Part model, mm, in its own coordinate system. A direction names the side the tool comes from. Coordinates: 2 decimals unless noted, no trailing zeros. Write each loop counter-clockwise with the first axis right and the second up, starting at its lowest first coordinate (ties: lowest second). Pieces come first, ordered by that corner, then holes. Notation, with made-up numbers: (81.5, 64) -> (136.5, 64) arc R27 cw to (136.5, 90) -> close; hole circle Ø4 at (21, 44.5). An arc over 180 degrees is marked (long way). Write item = value, one per line. Start each with the question number.
Q1. Band-saw the part on D-D, the plane x = 127. List the corners of the cut face in (y, z).
Q2. Band-saw the part on C-C, the plane x = 62. List the corners of the cut face in (y, z), plus the area to 3 significant figures.
Q3. Pull direction X, two halves, no side cores. Call faces 3 (the flat face through (45, 0, 0)), 4 (the cylindrical face through (25.344, 11.126, -19.936)), 5 (the cylindrical face through (66.6, 9.9, 35)): released by +X, released by -X, zero draft, split by the parting line, or undercut.
Q4. Pin check, flat tips, straight feed: P1, Ø5, axis at y = 13.5, z = 15.5, coming from the -X side; P2, Ø5, axis at x = 10.5, y = 7.5, coming from the -Z side; P3, Ø1.5, axis at x = 114, y = 17, coming from the +Z side; P4, Ø8, axis at x = 19, z = -3.5, coming from the -Y side. Stop position of each tip, or through.
Q5. Band-saw the part on A-A, the plane z = 0. List the corners of the cut face in (x, y), plus the area to 3 significant figures.
Q6. Band-saw the part on B-B, the plane y = 10.5. List the corners of the cut face in (x, z).
Q7. Tool access for faces 1 (the cylindrical face through (105.758, 11.126, 19.618)), 2 (the cylindrical face through (143.727, 0.986, -0.976)): list every direction of +Z, -Z, +X, -X, +Y, -Y with a clear straight run to the whole face (end or side of a thin tool).
Q8. Probe line 1 (X direction, y = 1.25, z = 0); line 2 (X direction, y = 7.5, z = 0); line 3 (Z direction, x = 64.5, y = 13). List the from-to ranges inside material, lowest first.
from build123d import *

# Parameters (mm, degrees)
PLATE_OUTLINE_AND_HOLES_SKETCH_R   = 7.5
PLATE_OUTLINE_AND_HOLES_SKETCH_R_2 = 20
PLATE_BODY_20MM_DEPTH              = 20
POCKET_18MM_DEEP_DEPTH             = 18


with BuildPart() as part:
    # Plate Outline and Holes Sketch → Plate Body 20mm (new body)
    with BuildSketch(Plane(origin=(0, 0, 0), x_dir=(1, 0, 0), z_dir=(0, 1, 0))):
        with BuildLine():
            ThreePointArc((0, -19.652996117), (25.514601751, -22.586747832), (49.820562895, -30.88265372))
            ThreePointArc((49.820562895, -30.88265372), (51.138080036, -31.506466617), (52.447922151, -32.146238124))
            ThreePointArc((52.447922151, -32.146238124), (66.786580153, -34.996485409), (81.03870417, -31.741030931))
            ThreePointArc((81.03870417, -31.741030931), (82.081542873, -31.206935864), (83.12954659, -30.683048174))
            ThreePointArc((83.12954659, -30.683048174), (105.326078872, -22.335617103), (128.730725009, -18.516168186))
            ThreePointArc((128.730725009, -18.516168186), (156.18959255, -2.007382475), (132.581174315, 19.652996117))
            ThreePointArc((132.581174315, 19.652996117), (106.605286262, 22.709869626), (81.908714055, 31.322102615))
            ThreePointArc((81.908714055, 31.322102615), (81.473287731, 31.530691668), (81.03870417, 31.741030931))
            ThreePointArc((81.03870417, 31.741030931), (66.786580153, 34.996485409), (52.447922151, 32.146238124))
            ThreePointArc((52.447922151, 32.146238124), (51.138080036, 31.506466617), (49.820562895, 30.88265372))
            ThreePointArc((49.820562895, 30.88265372), (25.514601751, 22.586747832), (0, 19.652996117))
            ThreePointArc((0, 19.652996117), (-23.709412843, 0), (0, -19.652996117))
        make_face()
        with Locations(Location((-3.709412843, 0, 0), (0, 0, 270))):
            Circle(PLATE_OUTLINE_AND_HOLES_SKETCH_R, mode=Mode.SUBTRACT)
        with Locations(Location((66.290587157, 0, 0), (0, 0, 270))):
            Circle(PLATE_OUTLINE_AND_HOLES_SKETCH_R_2, mode=Mode.SUBTRACT)
        with Locations(Location((136.290587157, 0, 0), (0, 0, 270))):
            Circle(PLATE_OUTLINE_AND_HOLES_SKETCH_R, mode=Mode.SUBTRACT)
    extrude(amount=PLATE_BODY_20MM_DEPTH)

    # Pocket Outline Sketch → Pocket 18mm Deep (cut)
    with BuildSketch(Plane(origin=(0, 20, 0), x_dir=(1, 0, 0), z_dir=(0, 1, 0))):
        with BuildLine():
            ThreePointArc((0, 16.772992409), (-20.887684525, 0), (0, -16.772992409))
            ThreePointArc((0, -16.772992409), (24.982456418, -19.938077439), (49.092914173, -27.206276583))
            ThreePointArc((49.092914173, -27.206276583), (66.290587157, -32.186044206), (83.488260142, -27.206276583))
            ThreePointArc((83.488260142, -27.206276583), (106.082407894, -19.537899767), (129.668226583, -15.931146045))
            ThreePointArc((129.668226583, -15.931146045), (153.543328212, 0), (129.668226583, 15.931146045))
            ThreePointArc((129.668226583, 15.931146045), (106.363417967, 20.688843047), (83.488260142, 27.206276583))
            ThreePointArc((83.488260142, 27.206276583), (66.290587157, 32.186044206), (49.092914173, 27.206276583))
            ThreePointArc((49.092914173, 27.206276583), (24.998686698, 19.861707266), (0, 16.772992409))
        make_face()
    extrude(amount=-POCKET_18MM_DEEP_DEPTH, mode=Mode.SUBTRACT)


solid = part.part
Ans:
q1.outline = (0, -19.83) -> (20, -19.83) -> (20, -16.38) -> (2, -16.38) -> (2, 16.13) -> (20, 16.13) -> (20, 18.64) -> (0, 18.64) -> close
q2.outline = (0, -34.74) -> (20, -34.74) -> (20, -31.9) -> (2, -31.9) -> (2, -19.53) -> (0, -19.53) -> close; (0, 19.53) -> (2, 19.53) -> (2, 31.9) -> (20, 31.9) -> (20, 34.74) -> (0, 34.74) -> close
q2.area = 163 mm2
q3.face_3 = zero draft
q3.face_4 = undercut
q3.face_5 = split by the parting line
q4.P1 = -18.91
q4.P2 = -20.45
q4.P3 = 20.51
q4.P4 = 0
q5.outline = (-23.71, 0) -> (-11.21, 0) -> (-11.21, 2) -> (-20.89, 2) -> (-20.89, 20) -> (-23.71, 20) -> close; (3.79, 0) -> (46.29, 0) -> (46.29, 2) -> (3.79, 2) -> close; (86.29, 0) -> (128.79, 0) -> (128.79, 2) -> (86.29, 2) -> close; (143.79, 0) -> (156.29, 0) -> (156.29, 20) -> (153.54, 20) -> (153.54, 2) -> (143.79, 2) -> close
q5.area = 320 mm2
q6.outline = (0, -19.65) arc R120 cw to (49.82, -30.88) arc R120 cw to (52.45, -32.15) arc R35 ccw to (81.04, -31.74) arc R120 cw to (81.91, -31.32) arc R120 cw to (132.58, -19.65) arc R20 ccw (long way) to (128.73, 18.52) arc R120 cw to (83.13, 30.68) arc R120 cw to (81.04, 31.74) arc R35 ccw to (52.45, 32.15) arc R120 cw to (49.82, 30.88) arc R120 cw to (0, 19.65) arc R20 ccw (long way) to start; hole (0, -16.77) arc R145.83 cw to (49.09, -27.21) arc R32.19 ccw to (83.49, -27.21) arc R312.32 cw to (129.67, -15.93) arc R17.25 ccw (long way) to (129.67, 15.93) arc R136.17 cw to (83.49, 27.21) arc R32.19 ccw to (49.09, 27.21) arc R151.17 cw to (0, 16.77) arc R17.18 ccw (long way) to start
q7.face_1 = +Y
q7.face_2 = +Y, -Y
q8.line_1 = -23.71 to -11.21, 3.79 to 46.29, 86.29 to 128.79, 143.79 to 156.29
q8.line_2 = -23.71 to -20.89, 153.54 to 156.29
q8.line_3 = -34.95 to -32.14, 32.14 to 34.95
